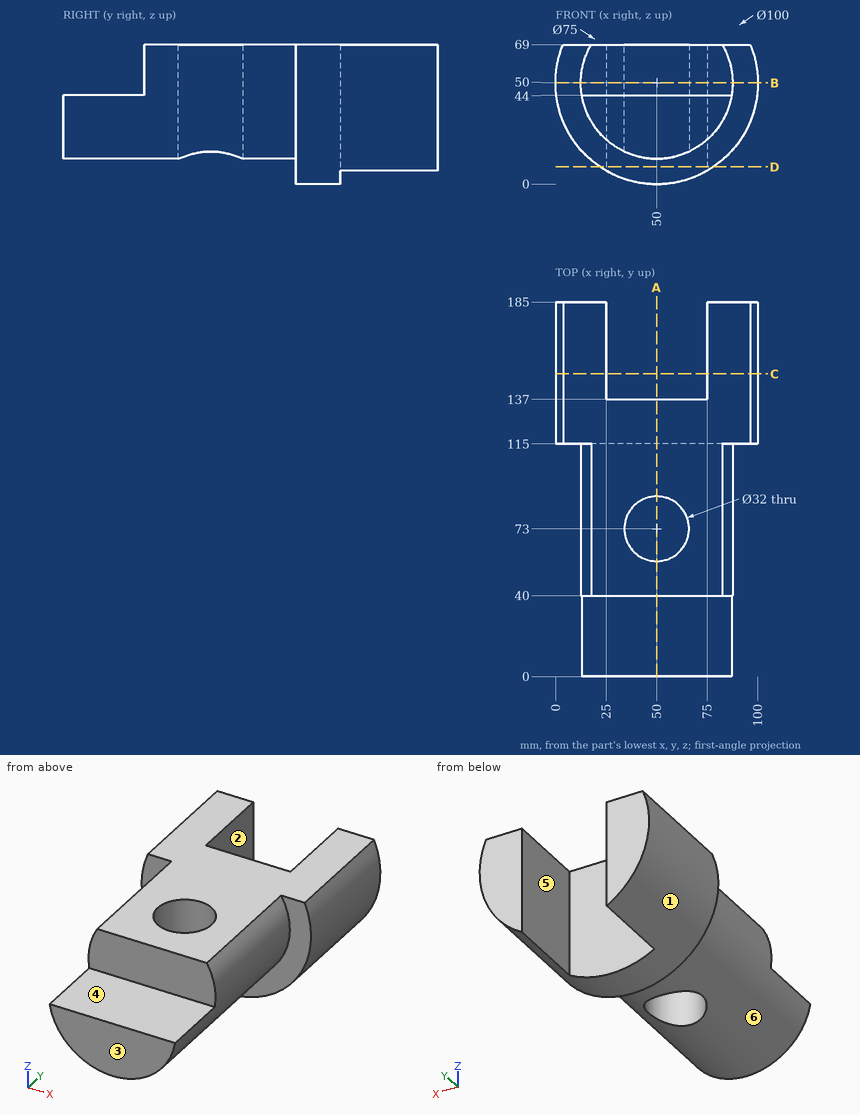
Could you check a few things on this drawing? It's one solid part, dimensions in mm from its lowest x, y, z. A direction names the side the tool comes from. Coordinates: 2 decimals unless noted, no trailing zeros. Order: outer loops, then holes, each group sorted by start corner. A loop starts at its lowest first (then second) coordinate and runs counter-clockwise, first axis right, second up. Notation, with made-up numbers: (15, 79.5) - (21, 79.5) arc R19 cw to (21, 88.5) - close; hole circle Ø3 at (-32.5, -36.75). An arc over 180 degrees is marked (long way). One line per question, with ' | ' between items. Start each with the question number.
1. Please list where these lines run through material, in increasing order: line 1 along Y through (x, z) = (50, 43); line 2 along Y through (x, z) = (77, 15); line 3 along Y through (x, z) = (47, 22). Write a range as [from, to].
2. If we section it at C-C (y = 149.5): Write out the boundary of the cut face in (x, z), and give its area (3 significant figures).
3. I'm going to push flat-ended pins straight in: pin 1 Ø5 at (y, z) = (74.5, 24) entering from -X; pin 2 Ø1 at (x, z) = (64.5, 49.5) entering from -Y; pin 3 Ø15 at (x, z) = (60.5, 49.5) entering from +Y; pin 4 Ø10 at (x, z) = (21, 48.5) entering from -Y. Where does each tip first touch, or does it pass through?
4. If we section it at D-D (z = 8.5): Write out the boundary of the cut face in (x, y).
5. If we section it at B-B (z = 50): Write out the boundary of the cut face in (x, y), and give its area (3 significant figures).
6. If we mould it in two halves opening along X, with no side actions, what happens to the marked faces 1, 2 and 3? For each: released by +X, released by -X, zero draft, split by the parting line, or undercut.
7. If we section it at A-A (x = 50): Write out the boundary of the cut face in (y, z), and give its area (3 significant figures).
8. Which directions (+Z, -Z, +X, -X, +Y, -Y) give clear straight access to the entire face, cutting with the end or side of a thin tool? Please do the marked faces 4, 5 and 6.
Model answer:
1) line 1: y = [0, 57], [89, 137] | line 2: y = [115, 185] | line 3: y = [0, 57.28], [88.72, 137]
2) outline: (3.75, 69) arc R50 ccw to (25, 6.7) - (25, 69) - close; (75, 6.7) arc R50 ccw to (96.25, 69) - (75, 69) - close | area: 2,440 mm²
3) pin 1: stops at x = 20.78 | pin 2: stops at y = 40 | pin 3: stops at y = 137 | pin 4: stops at y = 0
4) outline: (22.11, 115) - (77.89, 115) - (77.89, 185) - (75, 185) - (75, 137) - (25, 137) - (25, 185) - (22.11, 185) - close
5) outline: (0, 115) - (12.5, 115) - (12.5, 40) - (87.5, 40) - (87.5, 115) - (100, 115) - (100, 185) - (75, 185) - (75, 137) - (25, 137) - (25, 185) - (0, 185) - close; hole circle Ø32 at (50, 73) | area: 9,420 mm²
6) face 1: split by the parting line | face 2: undercut | face 3: zero draft
7) outline: (0, 12.5) - (57, 12.5) - (57, 69) - (40, 69) - (40, 44) - (0, 44) - close; (89, 12.5) - (115, 12.5) - (115, 0) - (137, 0) - (137, 69) - (89, 69) - close | area: 5,210 mm²
8) face 4: +Z, +X, -X, -Y | face 5: +Z, -Z, +Y | face 6: -Y
